from build123d import *

# Parameters (mm, degrees)
SKETCH2_W          = 1
SKETCH2_H          = 6.77698326
CUT_EXTRUDE1_DEPTH = 1


with BuildPart() as part:
    # Sketch1 → Revolve1 (revolve)
    with BuildSketch(Plane(origin=(0, 0, 0), x_dir=(1, 0, 0), z_dir=(0, 1, 0)), mode=Mode.PRIVATE) as revolve1_sk:
        Polygon((0, 0), (-10, 0), (-10, 1.6), (-9.7, 1.9), (-8, 1.9), (-8, 1.5), (-7, 1.5), (-7, 1.9), (-3.5, 1.9), (-3.5, 0.95), (-3, 0.95), (-3, 1.25), (-0.3, 1.25), (0, 0.95), align=None)
    revolve(revolve1_sk.sketch.rotate(Axis((0, 0, 0), (1, 0, 0)), 180), axis=Axis((0, 0, 0), (1, 0, 0)))

    # Sketch2 → Cut-Extrude1 (cut)
    with BuildSketch(Plane.ZY.offset(10)):
        Rectangle(SKETCH2_W, SKETCH2_H)
    extrude(amount=-CUT_EXTRUDE1_DEPTH, mode=Mode.SUBTRACT)


solid = part.part
Design review of the part built by this model. Coordinates are the model's own, in mm. A direction names the side the tool comes from. Coordinates: 2 decimals unless noted, no trailing zeros. Order: outer loops, then holes, each group sorted by start corner. A loop starts at its lowest first (then second) coordinate and runs counter-clockwise, first axis right, second up. Notation, with made-up numbers: M 61.25,54.25 L 86.25,54.25 A29 cw 86.25,78.25 Z; hole C -37,19.5 d10. An arc over 180 degrees is marked long. Use a Markdown table: item, result.
(1) Wall thickness on probe 1 along X at (y, z) = (-0.75, 1.4); probe 2 along X at (y, z) = (-1.6, 0.4); probe 3 along X at (y, z) = (0.7, 0.4): over which ranges is each line inside the solid? List them lowest first.
Worked answers:
| item | result |
|---|---|
| probe 1 | x = -10 to -8, -7 to -3.5 |
| probe 2 | x = -9 to -8, -7 to -3.5 |
| probe 3 | x = -9 to 0 |
(2) For P1, Ø0.5, axis at y = -0.5, z = 0, coming from the -X side; P2, Ø2, axis at x = -5, y = -1.5, coming from the +Z side, all flat-tipped, find the tip position at first contact; note any pin that passes through.
Worked answers:
| item | result |
|---|---|
| P1 | stops at x = -9 |
| P2 | stops at z = 1.83 |
(3) Add section D-D (x = -2.5). Give the boundary of the cut face in (y, z).
Worked answers:
| item | result |
|---|---|
| outline | C 0,0 d2.5 |
(4) For faces 5 (the cylindrical face through (-1.63, -0.05, -1.25)), 6 (the flat face through (-3.5, 1, 1)), 7 (the flat face through (-9, 0, 0)), 8 (the conical face through (-9.88, 0.03, 1.72)), list the 3-axis set-ups (+Z, -Z, +X, -X, +Y, -Y) from which the entire face can be reached by the end or side of a thin tool; tool diameter is ignored.
Worked answers:
| item | result |
|---|---|
| face 5 | +X |
| face 6 | none |
| face 7 | -X, +Y, -Y |
| face 8 | +Z, -X |
(5) Add section C-C (x = -4.5). Give the boundary of the cut face in (y, z), then the cut area to 3 significant figures.
Worked answers:
| item | result |
|---|---|
| outline | C 0,0 d3.8 |
| area | 11.3 mm2 |
(6) Add section B-B (y = 0). Give the boundary of the cut face in (x, z), then the cut area to 3 significant figures.
Worked answers:
| item | result |
|---|---|
| outline | M -10,-1.6 L -9.7,-1.9 L -8,-1.9 L -8,-1.5 L -7,-1.5 L -7,-1.9 L -3.5,-1.9 L -3.5,-0.95 L -3,-0.95 L -3,-1.25 L -0.3,-1.25 L 0,-0.95 L 0,0.95 L -0.3,1.25 L -3,1.25 L -3,0.95 L -3.5,0.95 L -3.5,1.9 L -7,1.9 L -7,1.5 L -8,1.5 L -8,1.9 L -9.7,1.9 L -10,1.6 L -10,0.5 L -9,0.5 L -9,-0.5 L -10,-0.5 Z |
| area | 31.2 mm2 |
(7) Draft analysis for pull direction X (two halves, no side actions). For faces 1 (the flat face through (-9.5, 0, -0.5)), 2 (the cylindrical face through (-7.49, -0.45, 1.43)), 3 (the conical face through (-9.88, -0.03, -1.72)), 4 (the flat face through (0, 0, 0)), state which applies: released by +X, released by -X, zero draft, split by the parting line, or undercut.
Worked answers:
| item | result |
|---|---|
| face 1 | zero draft |
| face 2 | undercut |
| face 3 | released by -X |
| face 4 | released by +X |
(8) Add section A-A (z = 0). Give the boundary of the cut face in (x, y).
Worked answers:
| item | result |
|---|---|
| outline | M -9,-1.9 L -8,-1.9 L -8,-1.5 L -7,-1.5 L -7,-1.9 L -3.5,-1.9 L -3.5,-0.95 L -3,-0.95 L -3,-1.25 L -0.3,-1.25 L 0,-0.95 L 0,0.95 L -0.3,1.25 L -3,1.25 L -3,0.95 L -3.5,0.95 L -3.5,1.9 L -7,1.9 L -7,1.5 L -8,1.5 L -8,1.9 L -9,1.9 Z |
